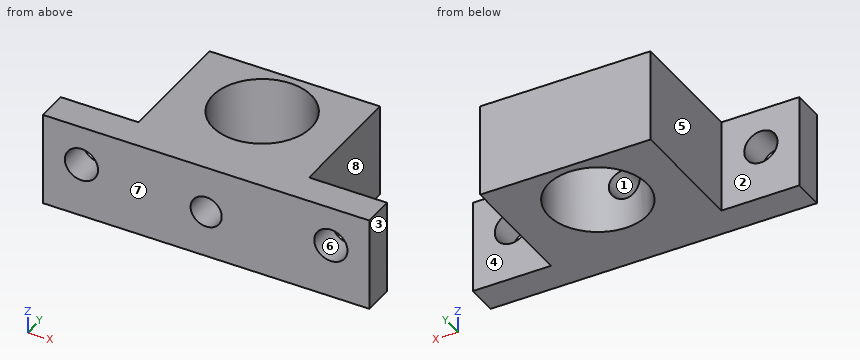
```python
from build123d import *

# Parameters (mm, degrees)
SKETCH1_W           = 40.4
SKETCH1_H           = 20
BOSS_EXTRUDE1_DEPTH = 15
SKETCH2_R           = 4.75
CUT_EXTRUDE1_DEPTH  = 36
SKETCH3_R           = 1.6
CUT_EXTRUDE2_DEPTH  = 36
SKETCH4_W           = 40.4
SKETCH4_H           = 8.8
CUT_EXTRUDE3_DEPTH  = 36
SKETCH5_W           = 40.4
SKETCH5_H           = 2.2
CUT_EXTRUDE4_DEPTH  = 36
SKETCH8_W           = 12
SKETCH8_H           = 9
CUT_EXTRUDE6_DEPTH  = 12
SKETCH10_W          = 4.5
SKETCH10_H          = 9
CUT_EXTRUDE7_DEPTH  = 12
SKETCH11_R          = 1.5
CUT_EXTRUDE8_DEPTH  = 10


with BuildPart() as part:
    # Sketch1 → Boss-Extrude1 (new body)
    with BuildSketch(Plane(origin=(0, 0, 0), x_dir=(1, 0, 0), z_dir=(0, 1, 0))):
        with Locations((20.2, -10)):
            Rectangle(SKETCH1_W, SKETCH1_H)
    extrude(amount=BOSS_EXTRUDE1_DEPTH)

    # Sketch2 → Cut-Extrude1 (cut)
    with BuildSketch(Plane.XY.offset(20)):
        with Locations((20.2, 9.5)):
            Circle(SKETCH2_R)
    extrude(amount=-CUT_EXTRUDE1_DEPTH, mode=Mode.SUBTRACT)

    # Sketch3 → Cut-Extrude2 (cut)
    with BuildSketch(Plane(origin=(0, 15, 0), x_dir=(1, 0, 0), z_dir=(0, 1, 0))):
        with Locations(Location((8.2, -14, 0), (0, 0, 270))):
            Circle(SKETCH3_R)
        with Locations(Location((32.2, -14, 0), (0, 0, 270))):
            Circle(SKETCH3_R)
    extrude(amount=-CUT_EXTRUDE2_DEPTH, mode=Mode.SUBTRACT)

    # Sketch4 → Cut-Extrude3 (cut)
    with BuildSketch(Plane(origin=(0, 15, 0), x_dir=(1, 0, 0), z_dir=(0, 1, 0))):
        with Locations((20.2, -4.4)):
            Rectangle(SKETCH4_W, SKETCH4_H)
    extrude(amount=-CUT_EXTRUDE3_DEPTH, mode=Mode.SUBTRACT)

    # Sketch5 → Cut-Extrude4 (cut)
    with BuildSketch(Plane(origin=(0, 15, 0), x_dir=(1, 0, 0), z_dir=(0, 1, 0))):
        with Locations((20.2, -18.9)):
            Rectangle(SKETCH5_W, SKETCH5_H)
    extrude(amount=-CUT_EXTRUDE4_DEPTH, mode=Mode.SUBTRACT)

    # Sketch8 → Cut-Extrude6 (cut)
    with BuildSketch(Plane(origin=(0, 15, 0), x_dir=(1, 0, 0), z_dir=(0, 1, 0))):
        with Locations((6, -13.3)):
            Rectangle(SKETCH8_W, SKETCH8_H)
        with Locations((34.4, -13.3)):
            Rectangle(SKETCH8_W, SKETCH8_H)
    extrude(amount=-CUT_EXTRUDE6_DEPTH, mode=Mode.SUBTRACT)

    # Sketch10 → Cut-Extrude7 (cut)
    with BuildSketch(Plane(origin=(0, 3, 0), x_dir=(1, 0, 0), z_dir=(0, 1, 0))):
        with Locations((2.25, -13.3)):
            Rectangle(SKETCH10_W, SKETCH10_H)
        with Locations((38.15, -13.3)):
            Rectangle(SKETCH10_W, SKETCH10_H)
    extrude(amount=-CUT_EXTRUDE7_DEPTH, mode=Mode.SUBTRACT)

    # Sketch11 → Cut-Extrude8 (cut)
    with BuildSketch(Plane.XZ):
        with Locations(Location((20.2, 13.3, 0), (0, 0, 270))):
            Circle(SKETCH11_R)
    extrude(amount=-CUT_EXTRUDE8_DEPTH, mode=Mode.SUBTRACT)


solid = part.part
```
The model under review builds one solid part; all positions refer to its coordinate system, in mm. Face numbers are marked on the shaded views. A direction names the side the tool comes from. Give positions to 0.01 mm unless a question says otherwise; leave off trailing zeros. Write each loop counter-clockwise with the first axis right and the second up, starting at its lowest first coordinate (ties: lowest second). Pieces come first, ordered by that corner, then holes. Notation, with made-up numbers: (40.5, 62) - (99.5, 62) arc R10 ccw to (99.5, 67) - close; hole circle Ø6 at (74, 16). An arc over 180 degrees is marked (long way). Answer in a Markdown table with one row per item. Add a question column.
1. We need section D-D on x = 32.2. Write out the cut boundary in (y, z), then the cut area to 3 significant figures.
2. We need section A-A on x = 20.2. Write out the cut boundary in (y, z).
3. Tool access review of the marked faces 1, 2, 3 and 4: name each direction out of +Z, -Z, +X, -X, +Y, -Y from which nothing blocks a thin tool from reaching the whole face with its end or side.
4. Insertion check: P1, Ø1, axis at y = 6, z = 11.5, coming from the +X side; P2, Ø2, axis at x = 9, z = 13.5, coming from the +Y side. Each pin has a flat end and moves straight along its axis. Give the tip position at first contact, or say it passes through.
5. We need section C-C on z = 16.5. Write out the cut boundary in (x, y).
6. Draft analysis for pull direction X (two halves, no side actions). For the marked faces 5, 6, 7 and 8, state which applies: +X half, -X half, draft (parallel to the pull), parting line (faces both ways), or undercut.
7. We need section B-B on y = 11. Write out the cut boundary in (x, z), then the cut area to 3 significant figures.
8. Wall thickness on line 1 along Z through (x, y) = (20.2, 2.35); line 2 along X through (y, z) = (0.95, 14); line 3 along Y through (x, z) = (34, 13.25): over which ranges is each line inside the solid? List them lowest first. Write a range as [from, to].
Ans:
| question | item | result |
|---|---|---|
| 1 | outline | (0, 8.8) - (3, 8.8) - (3, 12.4) - (0, 12.4) - close; (0, 15.6) - (3, 15.6) - (3, 17.8) - (0, 17.8) - close |
| 1 | area | 17.4 mm^2 |
| 2 | outline | (0, 8.8) - (4.75, 8.8) - (4.75, 11.8) - (0, 11.8) - close; (0, 14.8) - (4.75, 14.8) - (4.75, 17.8) - (0, 17.8) - close; (14.25, 8.8) - (15, 8.8) - (15, 17.8) - (14.25, 17.8) - close |
| 3 | face 1 | -Y |
| 3 | face 2 | +Z, -Z, -X, +Y |
| 3 | face 3 | +Z, -Z, +X, +Y, -Y |
| 3 | face 4 | +Z, -Z, +X, +Y |
| 4 | P1 | stops at x = 28.4 |
| 4 | P2 | stops at y = 3 |
| 5 | outline | (4.5, 0) - (35.9, 0) - (35.9, 3) - (28.4, 3) - (28.4, 15) - (12, 15) - (12, 3) - (4.5, 3) - close; hole circle Ø9.5 at (20.2, 9.5) |
| 6 | face 5 | -X half |
| 6 | face 6 | undercut |
| 6 | face 7 | draft |
| 6 | face 8 | +X half |
| 7 | outline | (12, 8.8) - (15.69, 8.8) - (15.69, 17.8) - (12, 17.8) - close; (24.71, 8.8) - (28.4, 8.8) - (28.4, 17.8) - (24.71, 17.8) - close |
| 7 | area | 66.5 mm^2 |
| 8 | line 1 | z = [8.8, 11.8], [14.8, 17.8] |
| 8 | line 2 | x = [4.5, 6.6], [9.8, 18.87], [21.53, 30.6], [33.8, 35.9] |
| 8 | line 3 | y = [0, 3] |
